Can you work these out from the model? Positions are in its coordinate system, mm. Coordinates: 2 decimals unless noted, no trailing zeros. Order: outer loops, then holes, each group sorted by start corner. A loop starts at its lowest first (then second) coordinate and runs counter-clockwise, first axis right, second up. Notation, with made-up numbers: (-5.5, 6.5) - (31.5, 6.5) arc R22 ccw to (31.5, 13.5) - close; hole circle Ø4 at (73, 1.5). An arc over 180 degrees is marked (long way). Use a Markdown table: item, result. Add a question column.
(1) I want a section at A-A (x = 10.5). List the corners of the cut face in (y, z) for me.
(2) If I drill on L1, parallel to Y at x = -10.5, z = -0.3; L2, parallel to X at y = 8, z = -1.2; L3, parallel to Y at x = -9.75, z = 0.85, over which ranges is the centre line in solid material (lowest first)? Write a range as [from, to].
(3) For pin 1 Ø2.5 at (x, y) = (-10.5, -7) entering from +Z, with a flat end and sliding along its axis, tell me the tip position at first contact or that it passes through.
(4) I want a section at C-C (y = -7). List the corners of the cut face in (x, z) for me.
(5) I want a section at B-B (z = -1). List the corners of the cut face in (x, y) for me.
(6) We'd pull the mould along X, two halves only. Please class faces 1 (the flat face through (14, 0, 0)), 2 (the cylindrical face through (-11.77, -7.97, -0.02)), 3 (the cylindrical face through (-9.23, 7.97, -0.02)), 4 (the flat face through (0, 0, -1.5)): pulls with the +X half, pulls with the -X half, needs draft (parallel to the pull), parting line crosses it, or undercut.
```python
from build123d import *

# Parameters (mm, degrees)
SKETCH1_W           = 28
SKETCH1_H           = 20
SKETCH1_R           = 1.6
BOSS_EXTRUDE1_DEPTH = 1.5


with BuildPart() as part:
    # Sketch1 → Boss-Extrude1 (new, symmetric)
    with BuildSketch(Plane.XY):
        Rectangle(SKETCH1_W, SKETCH1_H)
        with Locations((10.5, 7)):
            Circle(SKETCH1_R, mode=Mode.SUBTRACT)
        with Locations(Location((-10.5, 7, 0), (0, 0, 180))):
            Circle(SKETCH1_R, mode=Mode.SUBTRACT)
        with Locations(Location((10.5, -7, 0), (0, 0, 180))):
            Circle(SKETCH1_R, mode=Mode.SUBTRACT)
        with Locations((-10.5, -7)):
            Circle(SKETCH1_R, mode=Mode.SUBTRACT)
    extrude(amount=BOSS_EXTRUDE1_DEPTH, both=True)


solid = part.part
```
Answers follow:
| question | item | result |
|---|---|---|
| 1 | outline | (-10, -1.5) - (-8.6, -1.5) - (-8.6, 1.5) - (-10, 1.5) - close; (-5.4, -1.5) - (5.4, -1.5) - (5.4, 1.5) - (-5.4, 1.5) - close; (8.6, -1.5) - (10, -1.5) - (10, 1.5) - (8.6, 1.5) - close |
| 2 | L1 | y = [-10, -8.6], [-5.4, 5.4], [8.6, 10] |
| 2 | L2 | x = [-14, -11.75], [-9.25, 9.25], [11.75, 14] |
| 2 | L3 | y = [-10, -8.41], [-5.59, 5.59], [8.41, 10] |
| 3 | pin 1 | passes through |
| 4 | outline | (-14, -1.5) - (-12.1, -1.5) - (-12.1, 1.5) - (-14, 1.5) - close; (-8.9, -1.5) - (8.9, -1.5) - (8.9, 1.5) - (-8.9, 1.5) - close; (12.1, -1.5) - (14, -1.5) - (14, 1.5) - (12.1, 1.5) - close |
| 5 | outline | (-14, -10) - (14, -10) - (14, 10) - (-14, 10) - close; hole circle Ø3.2 at (-10.5, -7); hole circle Ø3.2 at (-10.5, 7); hole circle Ø3.2 at (10.5, -7); hole circle Ø3.2 at (10.5, 7) |
| 6 | face 1 | pulls with the +X half |
| 6 | face 2 | undercut |
| 6 | face 3 | undercut |
| 6 | face 4 | needs draft |
